Source: CAD feature listing. Evaluate the final solid. Frame: model axes, mm. Face numbers are marked on the shaded views. Give positions to 0.01 mm unless a question says otherwise; leave off trailing zeros. Write each loop counter-clockwise with the first axis right and the second up, starting at its lowest first coordinate (ties: lowest second). Pieces come first, ordered by that corner, then holes. Notation, with made-up numbers: M 11.5,45.5 L 51.5,45.5 A15 cw 51.5,51.5 Z; hole C -11.75,-6 d1. An arc over 180 degrees is marked long. Return JSON: item names as keys, results as strings.
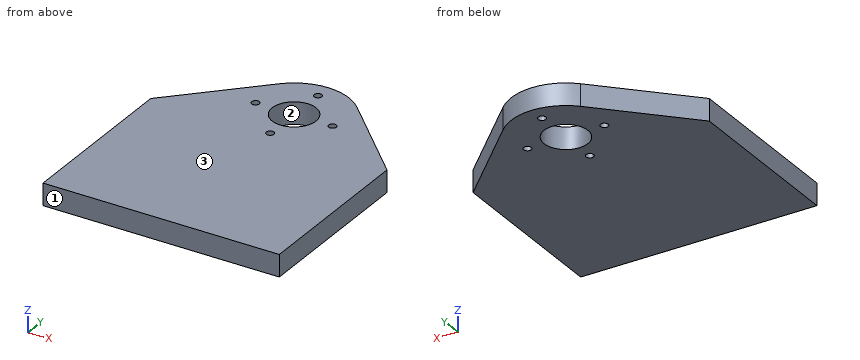
```python
from build123d import *

# Parameters (mm, degrees)
SKETCH1_R           = 40
BOSS_EXTRUDE1_DEPTH = 40
M16_TAPPED_HOLE1_D  = 14


with BuildPart() as part:
    # Sketch1 → Boss-Extrude1 (new body)
    with BuildSketch(Plane.XY):
        with BuildLine():
            Line((0, 0), (430.2, 0))
            Line((430.2, 0), (430.2, 316))
            Line((430.2, 316), (285.889255941, 460.632012878))
            ThreePointArc((285.889255941, 460.632012878), (215.1, 490), (144.310744059, 460.632012878))
            Line((144.310744059, 460.632012878), (0, 316))
            Line((0, 316), (0, 0))
        make_face()
        with Locations((215.1, 390)):
            Circle(SKETCH1_R, mode=Mode.SUBTRACT)
    extrude(amount=BOSS_EXTRUDE1_DEPTH)

    # M16 Tapped Hole1 (through all)
    with Locations(Plane.XY.offset(40)):
        with Locations((215.1, 460), (285.1, 390), (215.1, 320), (145.1, 390)):
            Hole(M16_TAPPED_HOLE1_D / 2)


solid = part.part
```
1) Draft query along Y for the marked faces 1, 2 and 3. Return one class per face: released by +Y, released by -Y, zero draft, split by the parting line, or undercut.
Numbers:
{"face 1": "released by -Y", "face 2": "undercut", "face 3": "zero draft"}
2) Contact query for flat-ended pins moving along their axis: pin 1 Ø22.5 at (x, y) = (145.1, 390) entering from +Z; pin 2 Ø5 at (y, z) = (378.5, 25) entering from +X; pin 3 Ø10 at (x, z) = (206, 15.5) entering from +Y. Output: stop coordinate, or through.
Numbers:
{"pin 1": "stops at z = 40", "pin 2": "stops at x = 370.33", "pin 3": "stops at y = 489.92"}
3) Line query: line 1 (Y direction, x = 215, z = 27); line 2 (X direction, y = 460, z = 25); line 3 (Y direction, x = 285.1, z = 29). Output: solid intervals per line, ascending. Write a range as [from, to].
Numbers:
{"line 1": "y = [0, 313], [327, 350], [430, 453], [467, 490]", "line 2": "x = [143.68, 208.1], [222.1, 286.52]", "line 3": "y = [0, 383], [397, 461.41]"}
4) Cut plane A-A, the plane x = 215.1. Return the cut outline in (y, z).
Numbers:
{"outline": "M 0,0 L 313,0 L 313,40 L 0,40 Z; M 327,0 L 350,0 L 350,40 L 327,40 Z; M 430,0 L 453,0 L 453,40 L 430,40 Z; M 467,0 L 490,0 L 490,40 L 467,40 Z"}
5) Cut plane C-C, the plane y = 390. Return the cut outline in (x, z), then the cut area to 3 significant figures.
Numbers:
{"outline": "M 73.84,0 L 138.1,0 L 138.1,40 L 73.84,40 Z; M 152.1,0 L 175.1,0 L 175.1,40 L 152.1,40 Z; M 255.1,0 L 278.1,0 L 278.1,40 L 255.1,40 Z; M 292.1,0 L 356.36,0 L 356.36,40 L 292.1,40 Z", "area": "6,980 mm²"}
6) Cut plane B-B, the plane z = 18. Return the cut outline in (x, y).
Numbers:
{"outline": "M 0,0 L 430.2,0 L 430.2,316 L 285.89,460.63 A100 ccw 144.31,460.63 L 0,316 Z; hole C 145.1,390 d14; hole C 215.1,390 d80; hole C 215.1,320 d14; hole C 215.1,460 d14; hole C 285.1,390 d14"}
7) Cut plane D-D, the plane x = 361.5. Return the cut outline in (y, z), then the cut area to 3 significant figures.
Numbers:
{"outline": "M 0,0 L 384.85,0 L 384.85,40 L 0,40 Z", "area": "15,400 mm²"}
